from build123d import *

# Parameters (mm, degrees)
BOSS_EXTRUDE1_DEPTH = 3
SKETCH3_R           = 3
CUT_EXTRUDE1_DEPTH  = 34.538336274
CHAMFER1_SIZE       = 1


with BuildPart() as part:
    # Sketch1 → Revolve1 (revolve)
    with BuildSketch(Plane.XY, mode=Mode.PRIVATE) as revolve1_sk:
        Polygon((0, 0), (5, 0), (5, -7), (6.7, -9), (6.7, -13.2), (6.25, -13.2), (6.25, -25.2), (8.7, -25.2), (8.7, -31.2), (0, -31.2), align=None)
    revolve(revolve1_sk.sketch.rotate(Axis((0, 0, 0), (0, -1, 0)), 90), axis=Axis((0, 0, 0), (0, -1, 0)))

    # Sketch2 → Boss-Extrude1 (add)
    with BuildSketch(Plane(origin=(0, -2, 0), x_dir=(1, 0, 0), z_dir=(0, 1, 0))):
        Polygon((-1.600084835, -6.506130073), (4.834431506, -4.638779152), (6.434516341, 1.867350921), (1.600084835, 6.506130073), (-4.834431506, 4.638779152), (-6.434516341, -1.867350921), align=None)
    extrude(amount=-BOSS_EXTRUDE1_DEPTH)

    # Sketch3 → Cut-Extrude1 (cut, through all)
    with BuildSketch(Plane(origin=(0, 0, 0), x_dir=(1, 0, 0), z_dir=(0, 1, 0))):
        with Locations(Location((0, 0, 0), (0, 0, 270))):
            Circle(SKETCH3_R)
    extrude(amount=-CUT_EXTRUDE1_DEPTH, mode=Mode.SUBTRACT)

    # Chamfer1
    chamfer1_edges = [part.edges().sort_by_distance(p)[0] for p in [
        (0, -25.2, -8.7),
    ]]
    chamfer(chamfer1_edges, length=CHAMFER1_SIZE)


solid = part.part
Model file for the job. Use its own axes, mm. A direction names the side the tool comes from. Round coordinates to 2 decimals unless told otherwise and drop trailing zeros. Order: outer loops, then holes, each group sorted by start corner. A loop starts at its lowest first (then second) coordinate and runs counter-clockwise, first axis right, second up.
(1) Band-saw the part on A-A (y = -4). List the corners of the cut face in (x, z).
(2) Band-saw the part on D-D (y = -29). List the corners of the cut face in (x, z), then the cut area to 3 significant figures.
(3) Pin check, flat tips, straight feed: pin 1 (4 mm diameter, centred on y = -16.5, z = 4, fed in from +X); pin 2 (6 mm diameter, centred on x = 0, y = -19, fed in from +Z); pin 3 (1.5 mm diameter, centred on x = 5, y = -5, fed in from +Z). Stop position of each tip, or through.
(4) 3-axis set-ups, long thin cutter, end or side, ignore diameter. For faces 4 (the face through (-4.051, -3.479, 4.154)), 5 (the face through (-5.623, -3.479, -1.431)), 6 (the face through (0, -1, -5)), 7 (the face through (-4.31, -7.13, 2.75)), 8 (the face through (4.051, -3.479, -4.154)): which of +Z, -Z, +X, -X, +Y, -Y reach the whole face in a straight line?
(5) Pull direction X, two halves, no side cores. Call faces 1 (the face through (-2, -5, 5)), 2 (the face through (0.9, -15.38, 2.86)), 3 (the face through (1.572, -3.479, 5.586)): released by +X, released by -X, zero draft, split by the parting line, or undercut.
(6) Drill centre lines: line 1 (X direction, y = -11, z = 0); line 2 (X direction, y = -21, z = 0); line 3 (Y direction, x = 5.75, z = -1.5). Where is each one in solid material? Low to high.
Verdict:
1. outline: (-6.43, 1.87) - (-4.83, -4.64) - (1.6, -6.51) - (6.43, -1.87) - (4.83, 4.64) - (-1.6, 6.51) - close; hole circle Ø6 at (0, 0)
2. outline: circle Ø17.4 at (0, 0); hole circle Ø6 at (0, 0)
2. area: 210 mm2
3. pin 1: stops at x = 5.92
3. pin 2: stops at z = 6.25
3. pin 3: stops at z = 4.81
4. face 4: +Z, -X, +Y
4. face 5: -Z, -X, +Y
4. face 6: +Y
4. face 7: none
4. face 8: -Z, +X, +Y
5. face 1: zero draft
5. face 2: undercut
5. face 3: released by +X
6. line 1: x = -6.7 to -3, 3 to 6.7
6. line 2: x = -6.25 to -3, 3 to 6.25
6. line 3: y = -31.2 to -8.11, -5 to -2
